Build history of the part. All positions in model axes, mm. Give positions to 0.01 mm unless a question says otherwise; leave off trailing zeros. Loops run counter-clockwise (first coordinate to the right, second up) from the corner with the lowest first, then second, coordinate; pieces in that order, holes last.
1) Wall check: line 1 (X direction, y = 10, z = 0.5); line 2 (Y direction, x = 1, z = 0); line 3 (Y direction, x = 3.5, z = -0.5). Give the ranges that are in metal, low to high.
2) Band-saw the part on B-B on y = 34. List the corners of the cut face in (x, z).
3) Band-saw the part on A-A on y = 7.5. List the corners of the cut face in (x, z).
```python
from build123d import *

# Parameters (mm, degrees)
SKETCH_1_R             = 4
EXTRUDE_1_DEPTH        = 70
CHAMFER_1_SIZE         = 0.5
HOLE_WIZARD_M4_1_D     = 3.3
HOLE_WIZARD_M4_1_DEPTH = 14.1
HOLE_WIZARD_M4_1_TIP   = 0.991420021


with BuildPart() as part:
    # 草图1 → 凸台-拉伸1 (new body)
    with BuildSketch(Plane(origin=(0, 0, 0), x_dir=(1, 0, 0), z_dir=(0, 1, 0))):
        with Locations(Location((0, 0, 0), (0, 0, 270))):
            Circle(SKETCH_1_R)
    extrude(amount=EXTRUDE_1_DEPTH)

    # 倒角1
    chamfer_1_edges = [part.edges().sort_by_distance(p)[0] for p in [
        (0, 0, -4),
        (0, 70, -4),
    ]]
    chamfer(chamfer_1_edges, length=CHAMFER_1_SIZE)

    # M4 螺纹孔1
    with Locations(Plane(origin=(0, 0, 0), x_dir=(-1, 0, 0), z_dir=(0, -1, 0))):
        with Locations((0, 0)):
            Hole(HOLE_WIZARD_M4_1_D / 2, depth=HOLE_WIZARD_M4_1_DEPTH)
            with Locations((0, 0, -(HOLE_WIZARD_M4_1_DEPTH + HOLE_WIZARD_M4_1_TIP / 2))):  # 118° drill point
                Cone(0, HOLE_WIZARD_M4_1_D / 2, HOLE_WIZARD_M4_1_TIP, mode=Mode.SUBTRACT)


solid = part.part
```
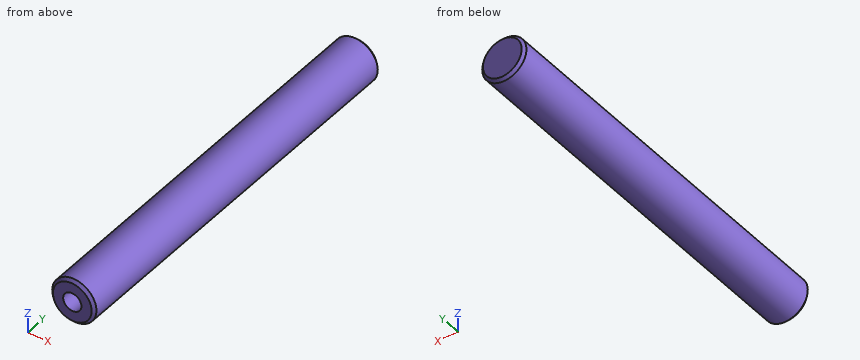
Findings below:
1. line 1: x = -3.97 to -1.57, 1.57 to 3.97
1. line 2: y = 14.49 to 70
1. line 3: y = 0.04 to 69.96
2. outline: circle Ø8 at (0, 0)
3. outline: circle Ø8 at (0, 0); hole circle Ø3.3 at (0, 0)
